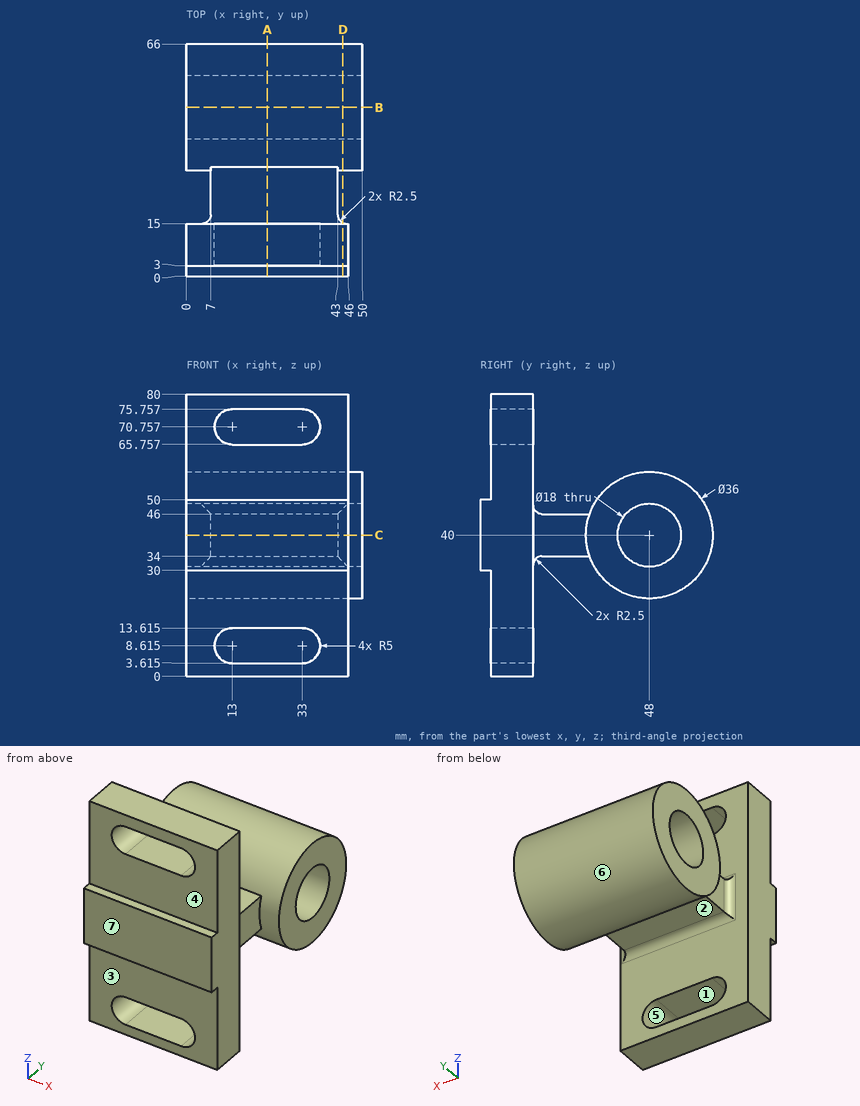
Study the drawing (mm; zero at the part's minimum x, y, z) and answer. A direction names the side the tool comes from. Coordinates: 2 decimals unless noted, no trailing zeros. Loops run counter-clockwise (first coordinate to the right, second up) from the corner with the lowest first, then second, coordinate; pieces in that order, holes last. Notation, with made-up numbers: (-4, 56) -> (37, 56) arc R17 ccw to (37, 81) -> close; hole circle Ø4 at (52.5, 26). An arc over 180 degrees is marked (long way). Answer in a Markdown table with one row per item. Add a question column.
1. The part is cut by section A-A, the plane x = 23. Write down the section's boundary in (y, z) (1 decimal).
2. The part is cut by section B-B, the plane y = 48. Write down the section's boundary in (x, z), then the cut area to 3 significant figures.
3. The part is cut by section D-D, the plane x = 44.5. Write down the section's boundary in (y, z).
4. Determine the mould class of the marked faces 5, 6 and 7 for opening direction Y: +Y half, -Y half, draft (parallel to the pull), parting line (faces both ways), or undercut.
5. For the marked faces 1, 2, 3 and 4, determine the directions among +Z, -Z, +X, -X, +Y, -Y from which every point of the face is accessible in a straight line to the end or side of a thin tool.
6. The part is cut by section C-C, the plane z = 40. Write down the section's boundary in (x, y), then the cut area to 3 significant figures.
7. Consider line 1 (Y direction, x = 33, z = 40); line 2 (Z direction, x = 35, y = 26.5); line 3 (Y direction, x = 13.5, z = 14). Determine where each line is inside the solid, lowest interval first. Write a range as [from, to].
8. Flat-ended cylindrical pins translate along their axes: P1, Ø9, axis at x = 18.5, z = 69, coming from the -Y side; P2, Ø5, axis at x = 26.5, y = 30.5, coming from the -Z side; P3, Ø12, axis at x = 7, y = 56, coming from the +Z side. Find the tip coordinate at first contact, or state that the pin passes through.
Answer below:
| question | item | result |
|---|---|---|
| 1 | outline | (0, 30) -> (3, 30) -> (3, 13.6) -> (15, 13.6) -> (15, 31.5) arc R2.5 cw to (17.5, 34) -> (31, 34) arc R18 ccw (long way) to (31, 46) -> (17.5, 46) arc R2.5 cw to (15, 48.5) -> (15, 65.8) -> (3, 65.8) -> (3, 50) -> (0, 50) -> close; (3, 0) -> (15, 0) -> (15, 3.6) -> (3, 3.6) -> close; (3, 75.8) -> (15, 75.8) -> (15, 80) -> (3, 80) -> close; hole circle Ø18 at (48, 40) |
| 2 | outline | (0, 22) -> (50, 22) -> (50, 31) -> (0, 31) -> close; (0, 49) -> (50, 49) -> (50, 58) -> (0, 58) -> close |
| 2 | area | 900 mm2 |
| 3 | outline | (0, 30) -> (3, 30) -> (3, 0) -> (15, 0) -> (15, 31.5) arc R2.5 cw to (15.21, 32.5) -> (15.21, 47.5) arc R2.5 cw to (15, 48.5) -> (15, 80) -> (3, 80) -> (3, 50) -> (0, 50) -> close; circle Ø36 at (48, 40); hole circle Ø18 at (48, 40) |
| 4 | face 5 | draft |
| 4 | face 6 | undercut |
| 4 | face 7 | -Y half |
| 5 | face 1 | +Y, -Y |
| 5 | face 2 | -Z, +X, -X |
| 5 | face 3 | -Z, +X, -X, -Y |
| 5 | face 4 | +Z, +X, -X, -Y |
| 6 | outline | (0, 0) -> (46, 0) -> (46, 15) -> (45.5, 15) arc R2.5 cw to (43, 17.5) -> (43, 30) -> (50, 30) -> (50, 39) -> (0, 39) -> (0, 30) -> (7, 30) -> (7, 17.5) arc R2.5 cw to (4.5, 15) -> (0, 15) -> close; (0, 57) -> (50, 57) -> (50, 66) -> (0, 66) -> close |
| 6 | area | 2,130 mm2 |
| 7 | line 1 | [0, 39], [57, 66] |
| 7 | line 2 | [34, 46] |
| 7 | line 3 | [3, 15] |
| 8 | P1 | y = 3 |
| 8 | P2 | z = 30.05 |
| 8 | P3 | z = 57.89 |
